For this review, take the finished solid that the model builds, in its own axes (mm). Face numbers are marked on the shaded views. Give positions to 0.01 mm unless a question says otherwise; leave off trailing zeros. Write each loop counter-clockwise with the first axis right and the second up, starting at its lowest first coordinate (ties: lowest second). Pieces come first, ordered by that corner, then holes. Notation, with made-up numbers: (-20.5, -27.75) -> (2.5, -27.75) arc R28 cw to (2.5, -3.75) -> close; hole circle Ø2 at (42, -30.75). An arc over 180 degrees is marked (long way). Write item = value, one per line.
```python
from build123d import *

# Parameters (mm, degrees)
SKETCH1_R           = 9
BOSS_EXTRUDE1_DEPTH = 20
SKETCH5_W           = 21
SKETCH5_H           = 16.784609691
CHAMFER1_SIZE       = 1


with BuildPart() as part:
    # Sketch1 → Boss-Extrude1 (new body)
    with BuildSketch(Plane.XY):
        with BuildLine():
            Line((26.69047619, 39.292091834), (62.614285714, 14.8896348))
            ThreePointArc((62.614285714, 14.8896348), (70.5, 0), (62.614285714, -14.8896348))
            Line((62.614285714, -14.8896348), (26.69047619, -39.292091834))
            ThreePointArc((26.69047619, -39.292091834), (0, -47.5), (-26.69047619, -39.292091834))
            Line((-26.69047619, -39.292091834), (-62.614285714, -14.8896348))
            ThreePointArc((-62.614285714, -14.8896348), (-70.5, 0), (-62.614285714, 14.8896348))
            Line((-62.614285714, 14.8896348), (-26.69047619, 39.292091834))
            ThreePointArc((-26.69047619, 39.292091834), (0, 47.5), (26.69047619, 39.292091834))
        make_face()
        with Locations((52.5, 0)):
            Circle(SKETCH1_R, mode=Mode.SUBTRACT)
        with Locations((-52.5, 0)):
            Circle(SKETCH1_R, mode=Mode.SUBTRACT)
    extrude(amount=BOSS_EXTRUDE1_DEPTH)

    # Sketch5 → Cut-Revolve1 (revolve, cut)
    with BuildSketch(Plane(origin=(0, 0, 0), x_dir=(1, 0, 0), z_dir=(0, 1, 0)), mode=Mode.PRIVATE) as cut_revolve1_sk:
        with Locations((10.5, -8.392304845)):
            Rectangle(SKETCH5_W, SKETCH5_H)
        Polygon((21, -16.784609691), (33, -20), (0, -20), (0, -16.784609691), align=None)
        Polygon((40, -20), (70.5, -20), (70.5, -17), align=None)
    revolve(cut_revolve1_sk.sketch.rotate(Axis((0, 0, 0), (0, 0, 1)), 180), axis=Axis((0, 0, 0), (0, 0, 1)), mode=Mode.SUBTRACT)

    # Chamfer1
    chamfer1_edges = [part.edges().sort_by_distance(p)[0] for p in [
        (21, 0, 0),
    ]]
    chamfer(chamfer1_edges, length=CHAMFER1_SIZE)


solid = part.part
```
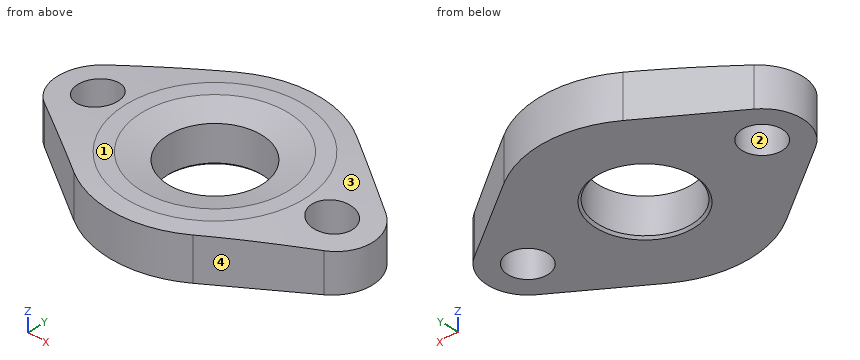
(1) Take a section at B-B (z = 14.25). Write out the cut boundary in (x, y).
Answers below:
outline = (-62.61, -14.89) -> (-26.69, -39.29) arc R47.5 ccw to (26.69, -39.29) -> (62.61, -14.89) arc R18 ccw to (62.61, 14.89) -> (26.69, 39.29) arc R47.5 ccw to (-26.69, 39.29) -> (-62.61, 14.89) arc R18 ccw to start; hole circle Ø18 at (-52.5, 0); hole circle Ø42 at (0, 0); hole circle Ø18 at (52.5, 0)
(2) The part is to be moulded in two halves that separate along Y. For the marked faces 1, 2, 3 and 4, say which applies: released by +Y, released by -Y, zero draft, split by the parting line, or undercut.
Answers below:
face_1 = zero draft
face_2 = undercut
face_3 = split by the parting line
face_4 = released by -Y
(3) To check wall thickness, follow probe 1 along X at (y, z) = (-5.5, 9); probe 2 along X at (y, z) = (7.5, 14); probe 3 along Y at (x, z) = (-7.5, 4.75). State the ranges of each line that lie inside material, in increasing order.
Answers below:
probe_1 = -69.64 to -59.62, -45.38 to -20.27, 20.27 to 45.38, 59.62 to 69.64
probe_2 = -68.86 to -57.47, -47.53 to -19.62, 19.62 to 47.53, 57.47 to 68.86
probe_3 = -46.9 to -19.62, 19.62 to 46.9
(4) For pin 1 (10 mm diameter, centred on y = -3.5, z = 8, fed in from +X); pin 2 (6 mm diameter, centred on x = -22.5, z = 7.5, fed in from -Y); pin 3 (6 mm diameter, centred on x = 21.5, z = 13.5, fed in from -Y); pin 4 (1 mm diameter, centred on x = 19, z = 5.5, fed in from +Y), all flat-tipped, find the tip position at first contact; note any pin that passes through.
Answers below:
pin_1 = 70.5
pin_2 = -43.31
pin_3 = -43.75
pin_4 = 43.75
(5) Take a section at C-C (y = 0). Write out the cut boundary in (x, z), plus the area to 3 significant figures.
Answers below:
outline = (-70.5, 0) -> (-61.5, 0) -> (-61.5, 17.89) -> (-70.5, 17) -> close; (-43.5, 0) -> (-22, 0) -> (-21, 1) -> (-21, 16.78) -> (-33, 20) -> (-40, 20) -> (-43.5, 19.66) -> close; (21, 1) -> (22, 0) -> (43.5, 0) -> (43.5, 19.66) -> (40, 20) -> (33, 20) -> (21, 16.78) -> close; (61.5, 0) -> (70.5, 0) -> (70.5, 17) -> (61.5, 17.89) -> close
area = 1,170 mm^2
(6) Take a section at A-A (x = 0). Write out the cut boundary in (y, z).
Answers below:
outline = (-47.5, 0) -> (-22, 0) -> (-21, 1) -> (-21, 16.78) -> (-33, 20) -> (-40, 20) -> (-47.5, 19.26) -> close; (21, 1) -> (22, 0) -> (47.5, 0) -> (47.5, 19.26) -> (40, 20) -> (33, 20) -> (21, 16.78) -> close
